Verification items for the finished model (mm, model axes). A direction names the side the tool comes from. Give positions to 0.01 mm unless a question says otherwise; leave off trailing zeros. Loops run counter-clockwise (first coordinate to the right, second up) from the corner with the lowest first, then second, coordinate; pieces in that order, holes last. Notation, with made-up numbers: (-3, -20.5) -> (16, -20.5) arc R25 cw to (16, 16.5) -> close; hole circle Ø8 at (29.5, 12). An arc over 180 degrees is marked (long way). Answer in a Markdown table with one row per item. Add a question column.
Q1. Section check A-A on z = 33. Enter the section's corners in (x, y).
Q2. Material ranges on probe 1 along Y at (x, z) = (48, 40); probe 2 along Z at (x, y) = (44.5, 2.5); probe 3 along Z at (x, y) = (57, 5) (3 decimals), recorded low to high.
Q3. Set-up check for faces 1 (the face through (55, 65, -5)), 2 (the face through (12, 65, 50)), 3 (the face through (35, 35, 20)), 4 (the face through (8, 15, -5)): record each of +Z, -Z, +X, -X, +Y, -Y from which the full face is reachable in a straight line by a thin tool's end or side.
Q4. Section check C-C on z = 44.5. Enter the section's corners in (x, y).
Q5. Gauge pin test, flat ends, axial feed: P1, Ø2, axis at x = 53, y = 4, coming from the -Z side; P2, Ø12, axis at x = 45.5, y = 39, coming from the +Z side. Record the tip position at first contact, or that the pin passes through.
Q6. Section check B-B on x = 25. Enter the section's corners in (y, z), and give its area (3 significant figures).
Q7. Section check D-D on x = 62. Enter the section's corners in (y, z).
Q8. Release check for a two-part mould opening along Y. For faces 5 (the face through (63, 55, -5)), 6 (the face through (35, 65, 58)), 7 (the face through (35, 55, 39)), 8 (the face through (35, -5, 31)) record: pulls with the +Y half, pulls with the -Y half, needs draft (parallel to the pull), parting line crosses it, or undercut.
```python
from build123d import *

# Parameters (mm, degrees)
BASE_PLATE_SKETCH_W          = 70
BASE_PLATE_SKETCH_H          = 70
BASE_PLATE_70X70_DEPTH       = 20
WEB_BLOCK_SKETCH_W           = 15
WEB_BLOCK_SKETCH_H           = 10
WEB_BLOCK_DEPTH              = 25
SIDE_BLOCK_A_SKETCH_W        = 15
SIDE_BLOCK_A_SKETCH_H        = 10
SIDE_BLOCK_A_DEPTH           = 25
SIDE_BLOCK_B_SKETCH_W        = 15
SIDE_BLOCK_B_SKETCH_H        = 10
SIDE_BLOCK_B_DEPTH           = 25
POCKET_CUT_A_SKETCH_W        = 10
POCKET_CUT_A_SKETCH_H        = 10
POCKET_CUT_A_DEPTH           = 70
POCKET_CUT_B_SKETCH_W        = 10
POCKET_CUT_B_SKETCH_H        = 10
POCKET_CUT_B_DEPTH           = 70
FLANGE_A_5MM_DEPTH           = 5
FLANGE_B_5MM_DEPTH           = 5
ROUNDED_TAB_A_DEPTH          = 20
ROUNDED_START                = -20
ROUNDED_TAB_B_DEPTH          = 20
TAB_SLOTS_8X30_THROUGH_DEPTH = 80


with BuildPart() as part:
    # Base Plate Sketch → Base Plate 70x70 (new body)
    with BuildSketch(Plane.XY):
        with Locations((35, 35)):
            Rectangle(BASE_PLATE_SKETCH_W, BASE_PLATE_SKETCH_H)
    extrude(amount=BASE_PLATE_70X70_DEPTH)

    # Web Block Sketch → Web Block (add)
    with BuildSketch(Plane.XZ):
        with Locations((7.5, -5)):
            Rectangle(WEB_BLOCK_SKETCH_W, WEB_BLOCK_SKETCH_H)
        with Locations((62.5, -5)):
            Rectangle(WEB_BLOCK_SKETCH_W, WEB_BLOCK_SKETCH_H)
    extrude(amount=-WEB_BLOCK_DEPTH)

    # Side Block A Sketch → Side Block A (add)
    with BuildSketch(Plane(origin=(0, 70, 0), x_dir=(1, 0, 0), z_dir=(0, 1, 0))):
        with Locations((7.5, 5)):
            Rectangle(SIDE_BLOCK_A_SKETCH_W, SIDE_BLOCK_A_SKETCH_H)
    extrude(amount=-SIDE_BLOCK_A_DEPTH)

    # Side Block B Sketch → Side Block B (add)
    with BuildSketch(Plane(origin=(0, 70, 0), x_dir=(1, 0, 0), z_dir=(0, 1, 0))):
        with Locations((62.5, 5)):
            Rectangle(SIDE_BLOCK_B_SKETCH_W, SIDE_BLOCK_B_SKETCH_H)
    extrude(amount=-SIDE_BLOCK_B_DEPTH)

    # Pocket Cut A Sketch → Pocket Cut A (cut)
    with BuildSketch(Plane(origin=(70, 0, 0), x_dir=(0, 0, -1), z_dir=(1, 0, 0))):
        with Locations((5, 50)):
            Rectangle(POCKET_CUT_A_SKETCH_W, POCKET_CUT_A_SKETCH_H)
    extrude(amount=-POCKET_CUT_A_DEPTH, mode=Mode.SUBTRACT)

    # Pocket Cut B Sketch → Pocket Cut B (cut)
    with BuildSketch(Plane(origin=(70, 0, 0), x_dir=(0, 0, -1), z_dir=(1, 0, 0))):
        with Locations((5, 20)):
            Rectangle(POCKET_CUT_B_SKETCH_W, POCKET_CUT_B_SKETCH_H)
    extrude(amount=-POCKET_CUT_B_DEPTH, mode=Mode.SUBTRACT)

    # Flange A Sketch → Flange A 5mm (add)
    with BuildSketch(Plane.XZ):
        Polygon((0, 20), (70, 20), (70, -10), (55, -10), (55, 0), (15, 0), (15, -10), (0, -10), align=None)
    extrude(amount=FLANGE_A_5MM_DEPTH)

    # Flange B Sketch → Flange B 5mm (add)
    with BuildSketch(Plane(origin=(0, 70, 0), x_dir=(1, 0, 0), z_dir=(0, 1, 0))):
        Polygon((0, -20), (70, -20), (70, 10), (55, 10), (55, 0), (15, 0), (15, 10), (0, 10), align=None)
    extrude(amount=FLANGE_B_5MM_DEPTH)

    # Rounded Tab A Sketch → Rounded Tab A (add)
    with BuildSketch(Plane.XZ.offset(5)):
        with BuildLine():
            Line((0, 20), (0, 50))
            ThreePointArc((0, 50), (5.857864376, 64.142135624), (20, 70))
            Line((20, 70), (50, 70))
            ThreePointArc((50, 70), (64.142135624, 64.142135624), (70, 50))
            Line((70, 50), (70, 20))
            Line((70, 20), (0, 20))
        make_face()
    extrude(amount=-ROUNDED_TAB_A_DEPTH)

    # Rounded Tab B Sketch → Rounded Tab B (add)
    with BuildSketch(Plane(origin=(0, 75, 0), x_dir=(1, 0, 0), z_dir=(0, 1, 0)).offset(ROUNDED_START)):
        with BuildLine():
            Line((0, -20), (0, -50))
            ThreePointArc((0, -50), (5.857864376, -64.142135624), (20, -70))
            Line((20, -70), (50, -70))
            ThreePointArc((50, -70), (64.142135624, -64.142135624), (70, -50))
            Line((70, -50), (70, -20))
            Line((70, -20), (0, -20))
        make_face()
    extrude(amount=ROUNDED_TAB_B_DEPTH)

    # Tab Slots Sketch → Tab Slots 8x30 Through (cut)
    with BuildSketch(Plane.XZ.offset(5)):
        with BuildLine():
            Line((20, 58), (50, 58))
            ThreePointArc((50, 58), (58, 50), (50, 42))
            Line((50, 42), (20, 42))
            ThreePointArc((20, 42), (12, 50), (20, 58))
        make_face()
    extrude(amount=-TAB_SLOTS_8X30_THROUGH_DEPTH, mode=Mode.SUBTRACT)


solid = part.part
```
Taken from the geometry:
| question | item | result |
|---|---|---|
| 1 | outline | (0, -5) -> (70, -5) -> (70, 15) -> (0, 15) -> close; (0, 55) -> (70, 55) -> (70, 75) -> (0, 75) -> close |
| 2 | probe 1 | y = -5 to 15, 55 to 75 |
| 2 | probe 2 | z = 0 to 42, 58 to 70 |
| 2 | probe 3 | z = -10 to 46.127, 53.873 to 68.735 |
| 3 | face 1 | -Z, +Y, -Y |
| 3 | face 2 | +Y, -Y |
| 3 | face 3 | +Z, +X, -X |
| 3 | face 4 | -Z, +X, -X |
| 4 | outline | (0, -5) -> (14.19, -5) -> (14.19, 15) -> (0, 15) -> close; (0, 55) -> (14.19, 55) -> (14.19, 75) -> (0, 75) -> close; (55.81, -5) -> (70, -5) -> (70, 15) -> (55.81, 15) -> close; (55.81, 55) -> (70, 55) -> (70, 75) -> (55.81, 75) -> close |
| 5 | P1 | stops at z = 0 |
| 5 | P2 | stops at z = 20 |
| 6 | outline | (-5, 0) -> (75, 0) -> (75, 42) -> (55, 42) -> (55, 20) -> (15, 20) -> (15, 42) -> (-5, 42) -> close; (-5, 58) -> (15, 58) -> (15, 70) -> (-5, 70) -> close; (55, 58) -> (75, 58) -> (75, 70) -> (55, 70) -> close |
| 6 | area | 2,960 mm² |
| 7 | outline | (-5, -10) -> (15, -10) -> (15, 0) -> (55, 0) -> (55, -10) -> (75, -10) -> (75, 66) -> (55, 66) -> (55, 20) -> (15, 20) -> (15, 66) -> (-5, 66) -> close |
| 8 | face 5 | undercut |
| 8 | face 6 | needs draft |
| 8 | face 7 | undercut |
| 8 | face 8 | pulls with the -Y half |
